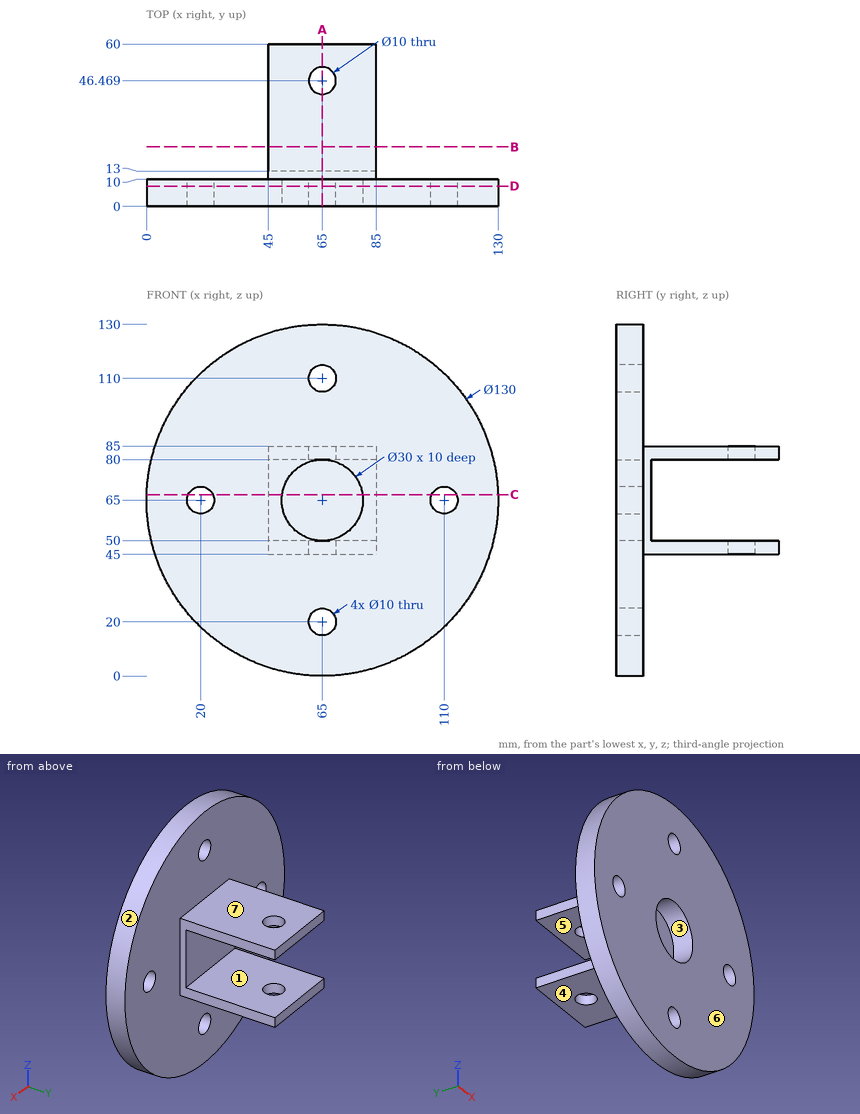
Part print with two shaded views. Sizes in mm from the minimum x, y, z corner. A direction names the side the tool comes from. Round coordinates to 2 decimals unless told otherwise and drop trailing zeros. Loops run counter-clockwise (first coordinate to the right, second up) from the corner with the lowest first, then second, coordinate; pieces in that order, holes last. Notation, with made-up numbers: M -6,28.25 L 33,28.25 A19 ccw 33,52.25 Z; hole C -8,26 d4. An arc over 180 degrees is marked long. Put each result on its own line as item: value. Start each with the question number.
Item 1: Drop flat-ended pins along their axis: P1, Ø15, axis at x = 75, z = 64, coming from the +Y side; P2, Ø4, axis at x = 41.5, z = 66.5, coming from the -Y side; P3, Ø6, axis at x = 110, z = 65, coming from the +Y side; P4, Ø4, axis at x = 31.5, z = 66, coming from the +Y side. Give the stop position or say it passes through.
Item 2: Cut at C-C (z = 67). List the corners of the cut face in (x, y), then the cut area to 3 significant figures.
Item 3: Cut at A-A (x = 65). Give the number of separate pieces and of enclosed holes in the cut face, then the cut area to 3 significant figures.
Item 4: Cut at B-B (y = 22). List the corners of the cut face in (x, z).
Item 5: Mould opens along Z. For the marked faces 5, 6 and 7 say: released by +Z, released by -Z, zero draft, split by the parting line, or undercut.
Item 6: 3-axis set-ups, long thin cutter, end or side, ignore diameter. For the marked faces 1, 2, 3 and 4: which of +Z, -Z, +X, -X, +Y, -Y reach the whole face in a straight line?
Item 7: Cut at D-D (y = 7.5). List the corners of the cut face in (x, z).
Item 8: Drill centre lines: line 1 along X through (y, z) = (4.5, 65); line 2 along Y through (x, z) = (65, 48.1); line 3 along Z through (x, y) = (65.5, 17.5). Where is each one in solid material? Low to high.
Answer block:
1. P1: y = 13
1. P2: y = 0
1. P3: through
1. P4: y = 10
2. outline: M 0.03,0 L 15.42,0 L 15.42,10 L 0.03,10 Z; M 24.58,0 L 50.13,0 L 50.13,10 L 79.87,10 L 79.87,0 L 105.42,0 L 105.42,10 L 85,10 L 85,13 L 45,13 L 45,10 L 24.58,10 Z; M 114.58,0 L 129.97,0 L 129.97,10 L 114.58,10 Z
2. area: 939 mm2
3. separate pieces: 5
3. enclosed holes: 0
3. area: 1,290 mm2
4. outline: M 45,45 L 85,45 L 85,50 L 45,50 Z; M 45,80 L 85,80 L 85,85 L 45,85 Z
5. face 5: undercut
5. face 6: zero draft
5. face 7: released by +Z
6. face 1: +X, -X, +Y
6. face 2: +Y, -Y
6. face 3: -Y
6. face 4: -Z, +X, -X, +Y
7. outline: C 65,65 d130; hole C 20,65 d10; hole C 65,65 d30; hole C 65,20 d10; hole C 65,110 d10; hole C 110,65 d10
8. line 1: 0 to 15, 25 to 50, 80 to 105, 115 to 130
8. line 2: 0 to 41.47, 51.47 to 60
8. line 3: 45 to 50, 80 to 85
